from build123d import *

# Parameters (mm, degrees)
SKETCH_1_R               = 60
SKETCH_1_R_2             = 50
EXTRUDE_1_DEPTH          = 20
SKETCH_2_R               = 3
CUT_EXTRUDE_1_DEPTH      = 88.177978871
PATTERN_CIRCULAR_1_COUNT = 6


with BuildPart() as part:
    # 草图1 → 凸台-拉伸1 (new body)
    with BuildSketch(Plane(origin=(0, 0, 0), x_dir=(1, 0, 0), z_dir=(0, 1, 0))):
        with Locations(Location((0, 0, 0), (0, 0, 270))):
            Circle(SKETCH_1_R)
        with Locations(Location((0, 0, 0), (0, 0, 270))):
            Circle(SKETCH_1_R_2, mode=Mode.SUBTRACT)
    extrude(amount=EXTRUDE_1_DEPTH)

    # 草图2 → 切除-拉伸1 (cut, through all)
    with BuildSketch(Plane(origin=(0, 20, 0), x_dir=(1, 0, 0), z_dir=(0, 1, 0))):
        with Locations(Location((0, 55, 0), (0, 0, 270))):
            Circle(SKETCH_2_R)
    cut_extrude_1 = extrude(amount=-CUT_EXTRUDE_1_DEPTH, mode=Mode.SUBTRACT)

    # 阵列(圆周)1: 切除-拉伸1 ×6 about axis
    pattern_circular_1_axis = Axis((0, 0, 0), (0, 1, 0))
    for i in range(1, PATTERN_CIRCULAR_1_COUNT):
        add(cut_extrude_1.rotate(pattern_circular_1_axis, i * 360 / PATTERN_CIRCULAR_1_COUNT), mode=Mode.SUBTRACT)


solid = part.part
Source: CAD feature listing. Evaluate the final solid. Frame: model axes, mm. Coordinates: 2 decimals unless noted, no trailing zeros. Loops run counter-clockwise (first coordinate to the right, second up) from the corner with the lowest first, then second, coordinate; pieces in that order, holes last. Notation, with made-up numbers: (70.25, 44.25) - (100.25, 44.25) arc R24 ccw to (100.25, 81.25) - close; hole circle Ø11 at (40, -13.75). An arc over 180 degrees is marked (long way). One line per item, written item: value. Start each with the question number.
1. Section A-A (x = 0). Return the cut outline in (y, z).
2. Contact query for flat-ended pins moving along their axis: P1, Ø2, axis at y = 14, z = 37.5, coming from the +X side; P2, Ø8, axis at y = 2, z = 23.5, coming from the -X side; P3, Ø5, axis at x = 0, z = 55, coming from the +Y side; P4, Ø10, axis at y = 8, z = -28.5, coming from the +X side. Output: stop coordinate, or through.
3. Section C-C (x = 21). Return the cut outline in (y, z), and give its area (3 significant figures).
4. Ray query, L1, parallel to X at y = 12.5, z = 0; L2, parallel to X at y = 6, z = -27.5; L3, parallel to Z at x = 45, y = 15.5. Return the intervals inside material, ascending.
5. Mould query, pull axis X, two halves, no side actions, for faces 1 (the flat face through (-49, 20, -14)), 2 (the cylindrical face through (2.64, 9.86, -59.94)), 3 (the cylindrical face through (50.56, 10.14, -26.85)), 4 (the cylindrical face through (0, 10, -58)). Classes: pulls with the +X half, pulls with the -X half, needs draft (parallel to the pull), parting line crosses it, or undercut.
6. Section B-B (z = 0). Return the cut outline in (x, y).
7. Section D-D (y = 11.75). Return the cut outline in (x, z), and give its area (3 significant figures).
Verdict:
1. outline: (0, -60) - (20, -60) - (20, -58) - (0, -58) - close; (0, -52) - (20, -52) - (20, -50) - (0, -50) - close; (0, 50) - (20, 50) - (20, 52) - (0, 52) - close; (0, 58) - (20, 58) - (20, 60) - (0, 60) - close
2. P1: stops at x = 47.62
2. P2: stops at x = -56.74
2. P3: passes through
2. P4: stops at x = 55.21
3. outline: (0, -56.2) - (20, -56.2) - (20, -45.38) - (0, -45.38) - close; (0, 45.38) - (20, 45.38) - (20, 56.2) - (0, 56.2) - close
3. area: 433 mm2
4. L1: x = -60 to -50, 50 to 60
4. L2: x = -53.33 to -50.63, -44.63 to -41.76, 41.76 to 44.63, 50.63 to 53.33
4. L3: z = -39.69 to -28.94, -26.06 to -21.79, 21.79 to 26.06, 28.94 to 39.69
5. face 1: needs draft
5. face 2: parting line crosses it
5. face 3: undercut
5. face 4: undercut
6. outline: (-60, 0) - (-50, 0) - (-50, 20) - (-60, 20) - close; (50, 0) - (60, 0) - (60, 20) - (50, 20) - close
7. outline: circle Ø120 at (0, 0); hole circle Ø6 at (-47.63, -27.5); hole circle Ø6 at (-47.63, 27.5); hole circle Ø100 at (0, 0); hole circle Ø6 at (0, -55); hole circle Ø6 at (0, 55); hole circle Ø6 at (47.63, -27.5); hole circle Ø6 at (47.63, 27.5)
7. area: 3,290 mm2
